Could you check a few things on this drawing? It's one solid part, dimensions in mm from its lowest x, y, z. A direction names the side the tool comes from. Give positions to 0.01 mm unless a question says otherwise; leave off trailing zeros. Loops run counter-clockwise (first coordinate to the right, second up) from the corner with the lowest first, then second, coordinate; pieces in that order, holes last.
1. Imagine slicing it at B-B (y = 21.5). List the corners of the cut face in (x, z) for me.
2. For the marked faces 1, 2 and 3, which set-ups out of +Z, -Z, +X, -X, +Y, -Y let a thin tool reach every point of the face, with its end or its side?
3. Imagine slicing it at A-A (y = 4). List the corners of the cut face in (x, z) for me.
4. I need wall thicknesses on line 1 along Z through (x, y) = (8, 15.5); line 2 along Y through (x, z) = (3.5, 12.25); line 3 along X through (y, z) = (5, 9.25) (1 decimal). Which ranges of each line are inside material? Lowest first, please.
5. Thinking about a two-plate mould opening in Y: for the marked faces 4, 5, 6 and 7, which applies, +Y half, -Y half, draft (parallel to the pull), parting line (faces both ways), or undercut?
6. For P1, Ø6, axis at x = 8.5, y = 3, coming from the +Z side; P2, Ø5, axis at x = 7, z = 9, coming from the -Y side; P3, Ø6, axis at y = 23.5, z = 5, coming from the -X side; P4, Ø4, axis at x = 12.5, y = 27.5, coming from the -Z side, each with a flat end and sliding along its axis, tell me the tip position at first contact or that it passes through.
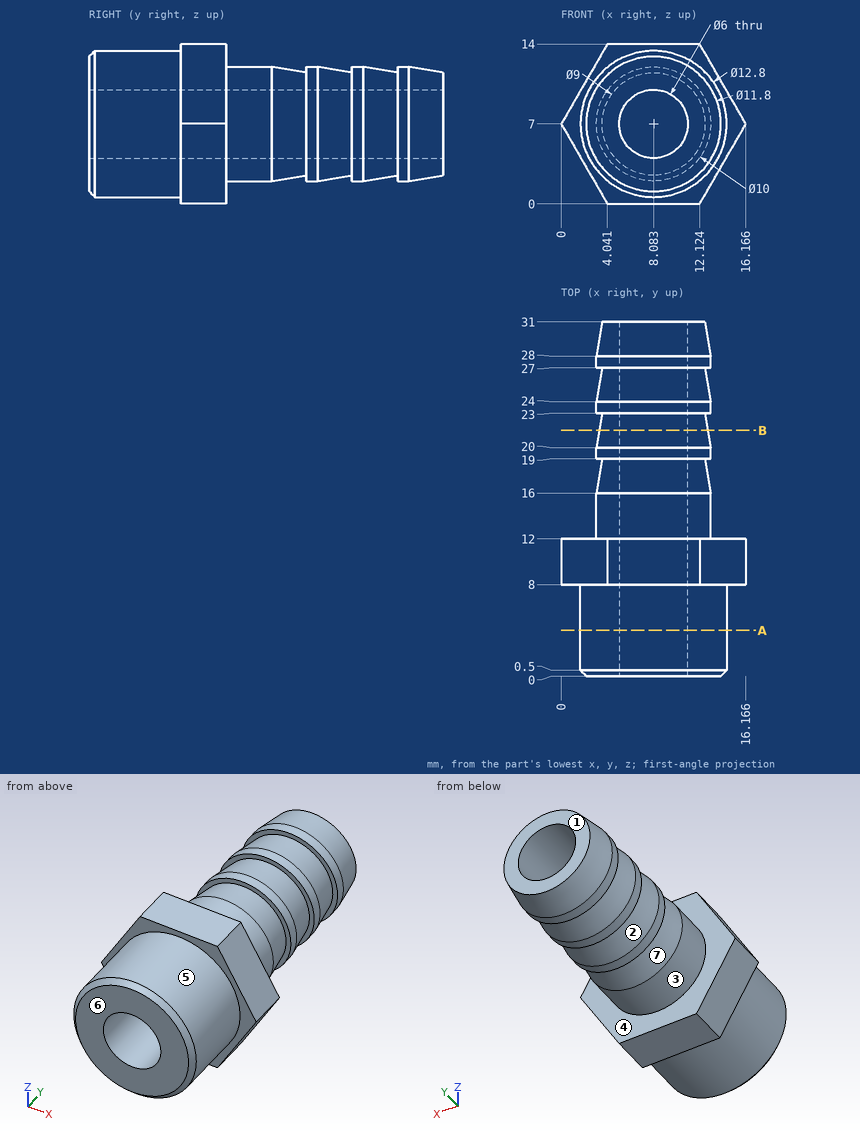
Derived:
1. outline: circle Ø9.5 at (8.08, 7); hole circle Ø6 at (8.08, 7)
2. face 1: +Z, -Z, +X, -X, +Y
2. face 2: none
2. face 3: +Y
3. outline: circle Ø12.8 at (8.08, 7); hole circle Ø6 at (8.08, 7)
4. line 1: z = 2 to 4, 10 to 12
4. line 2: y = 8 to 12
4. line 3: x = 2.1 to 6.1, 10.1 to 14.1
5. face 4: +Y half
5. face 5: draft
5. face 6: -Y half
5. face 7: undercut
6. P1: stops at z = 13.4
6. P2: stops at y = 0
6. P3: stops at x = 3.08
6. P4: stops at z = 2.62
